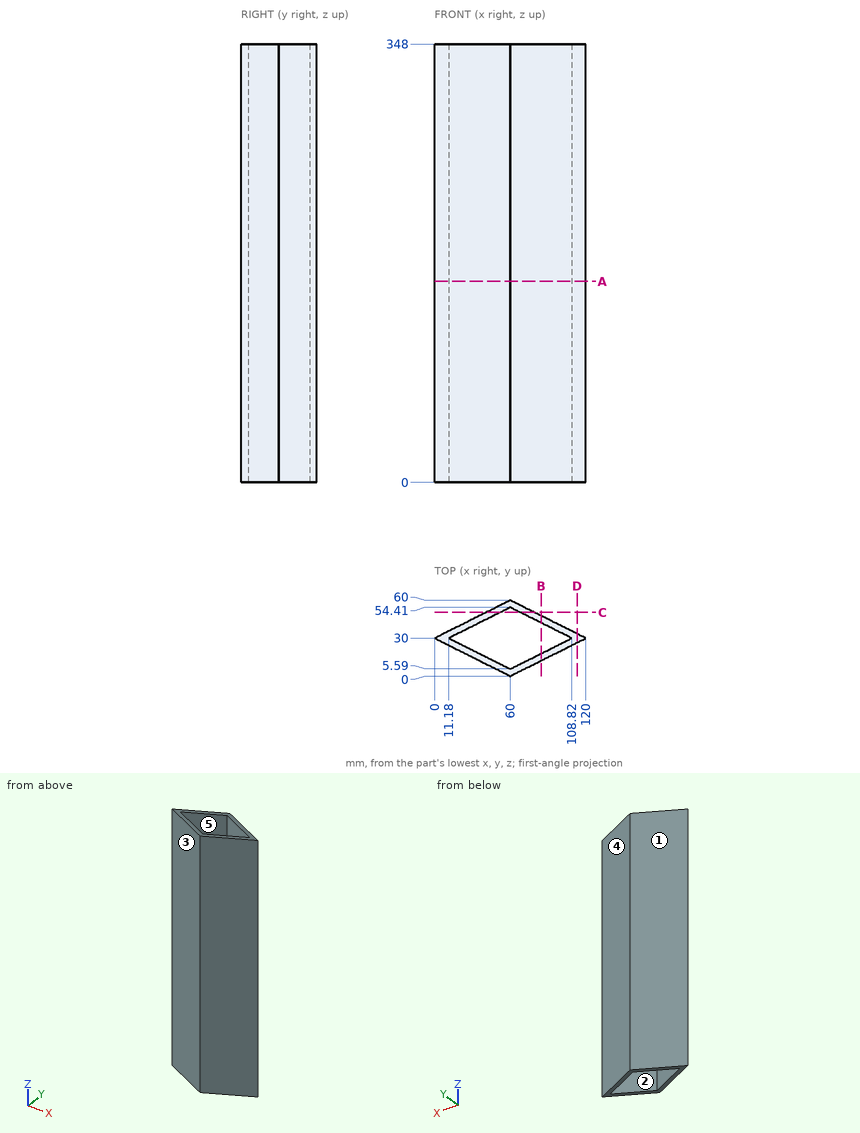
The figure shows three views and two pictorial views of one solid part (mm, origin at its lowest corner). Answer the questions. A direction names the side the tool comes from. Give positions to 0.01 mm unless a question says otherwise; leave off trailing zeros. Write each loop counter-clockwise with the first axis right and the second up, starting at its lowest first coordinate (ties: lowest second). Pieces come first, ordered by that corner, then holes. Notation, with made-up numbers: M 53,27 L 79,27 A17 cw 79,42 Z; hole C 22,-5.75 d10. An arc over 180 degrees is marked long. One line per item, written item: value. Start each with the question number.
(1) A tool of negligible diameter and unlimited length cuts with its end or side. For the marked faces 1 and 2, from which of +Z, -Z, +X, -X, +Y, -Y can it reach the whole face along a straight path? Write none if from no direction.
(2) Find section C-C (y = 50.5). Determine the outline of the cut face in (x, z).
(3) Find section D-D (x = 113). Determine the outline of the cut face in (y, z), plus the area to 3 significant figures.
(4) Find section B-B (x = 84.5). Determine the outline of the cut face in (y, z), plus the area to 3 significant figures.
(5) Find the intervals of material crossed by line 1 (X direction, y = 35, z = 328.5); line 2 (X direction, y = 30.5, z = 132); line 3 (Y direction, x = 67, z = 187.5), in increasing order.
(6) Flat-ended cylindrical pins translate along their axes: pin 1 Ø5 at (y, z) = (16, 174) entering from -X; pin 2 Ø3 at (x, z) = (18.5, 81.5) entering from -Y; pin 3 Ø6 at (x, z) = (13, 308.5) entering from -Y. Find the tip coordinate at first contact, or state that the pin passes through.
(7) Determine the mould class of the marked faces 3, 4 and 5 for opening direction Y: pulls with the +Y half, pulls with the -Y half, needs draft (parallel to the pull), parting line crosses it, or undercut.
(8) Find section A-A (z = 159.5). Determine the outline of the cut face in (x, y).
Results below:
1. face 1: +Z, -Z, -X, +Y
1. face 2: +Z, -Z
2. outline: M 41,0 L 52.18,0 L 52.18,348 L 41,348 Z; M 67.82,0 L 79,0 L 79,348 L 67.82,348 Z
3. outline: M 26.5,0 L 33.5,0 L 33.5,348 L 26.5,348 Z
3. area: 2,440 mm^2
4. outline: M 12.25,0 L 17.84,0 L 17.84,348 L 12.25,348 Z; M 42.16,0 L 47.75,0 L 47.75,348 L 42.16,348 Z
4. area: 3,890 mm^2
5. line 1: x = 10 to 21.18, 98.82 to 110
5. line 2: x = 1 to 12.18, 107.82 to 119
5. line 3: y = 3.5 to 9.09, 50.91 to 56.5
6. pin 1: stops at x = 23
6. pin 2: stops at y = 20
6. pin 3: stops at y = 22
7. face 3: pulls with the -Y half
7. face 4: pulls with the +Y half
7. face 5: undercut
8. outline: M 0,30 L 60,0 L 120,30 L 60,60 Z; hole M 11.18,30 L 60,5.59 L 108.82,30 L 60,54.41 Z
